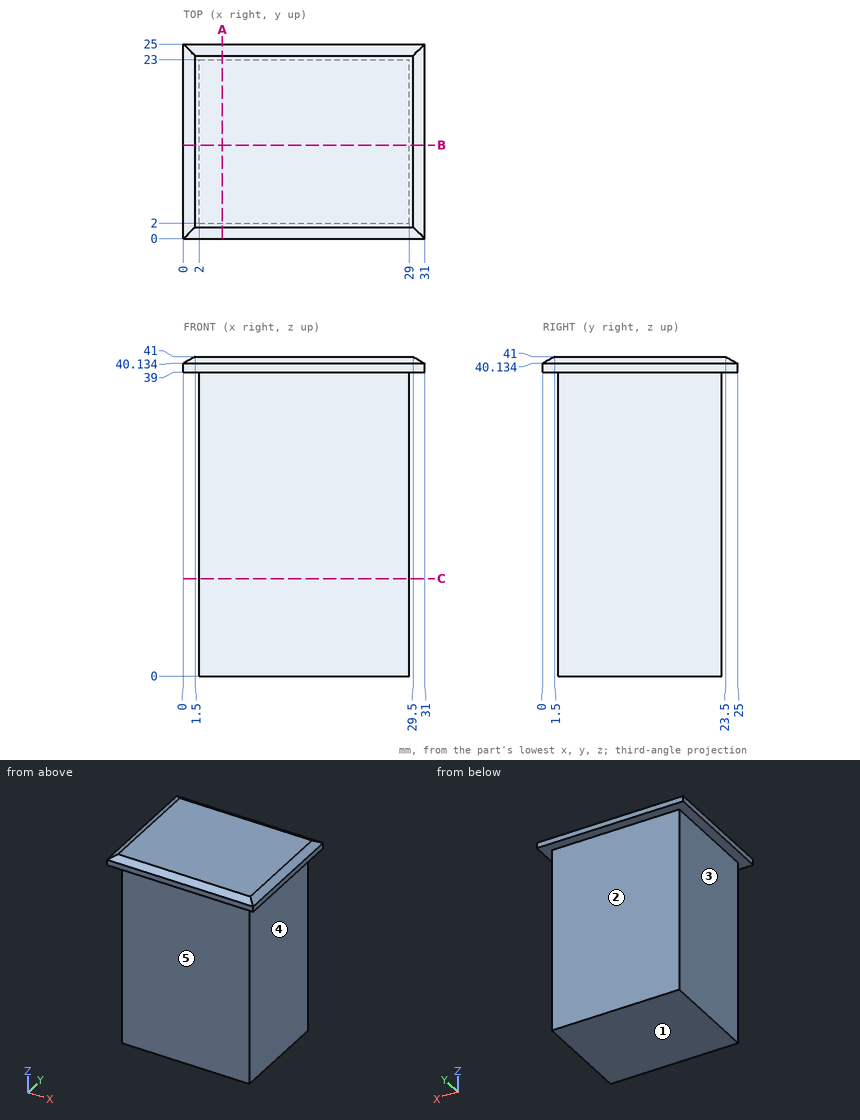
Check sheet for the drawn part. Datum: minimum x, y, z corner. Units: mm. A direction names the side the tool comes from. Round coordinates to 2 decimals unless told otherwise and drop trailing zeros. Loops run counter-clockwise (first coordinate to the right, second up) from the corner with the lowest first, then second, coordinate; pieces in that order, holes last. Notation, with made-up numbers: (-23.75, 63) -> (28.25, 63) arc R20 ccw to (28.25, 97) -> close; hole circle Ø4 at (-27.75, -9). An arc over 180 degrees is marked (long way). Put each result on its own line as item: value. Start each with the question number.
1. Section check B-B (y = 12). Enter the section's corners in (x, z), plus the area to 3 significant figures.
2. Access from +Z, -Z, +X, -X, +Y, -Y to the whole of each face (thin tool, end or side, straight path). Record for the marked faces 1, 2, 3, 4 and 5.
3. Gauge pin test, flat ends, axial feed: pin 1 (3 mm diameter, centred on x = 18.5, z = 22, fed in from +Y); pin 2 (13.5 mm diameter, centred on x = 21, z = 13.5, fed in from -Y); pin 3 (3 mm diameter, centred on y = 18, z = 32, fed in from +X). Record the tip position at first contact, or that the pin passes through.
4. Section check A-A (x = 5). Enter the section's corners in (y, z), plus the area to 3 significant figures.
5. Section check C-C (z = 12.5). Enter the section's corners in (x, y).
6. Scan lines: probe 1 along X at (y, z) = (11, 29.5); probe 2 along Y at (x, z) = (20.5, 35); probe 3 along Z at (x, y) = (10, 23.25). Record each from-to range of solid material in increasing order.
Findings:
1. outline: (0, 39) -> (2, 39) -> (2, 0) -> (29, 0) -> (29, 39) -> (31, 39) -> (31, 40.13) -> (29.5, 41) -> (1.5, 41) -> (0, 40.13) -> close
1. area: 1,110 mm^2
2. face 1: -Z, +X, -X, +Y, -Y
2. face 2: -Z, +X, -X, +Y
2. face 3: -Z, -X, +Y, -Y
2. face 4: -Z, +X, +Y, -Y
2. face 5: -Z, +X, -X, -Y
3. pin 1: stops at y = 23
3. pin 2: stops at y = 2
3. pin 3: stops at x = 29
4. outline: (0, 39) -> (2, 39) -> (2, 0) -> (23, 0) -> (23, 39) -> (25, 39) -> (25, 40.13) -> (23.5, 41) -> (1.5, 41) -> (0, 40.13) -> close
4. area: 868 mm^2
5. outline: (2, 2) -> (29, 2) -> (29, 23) -> (2, 23) -> close
6. probe 1: x = 2 to 29
6. probe 2: y = 2 to 23
6. probe 3: z = 39 to 41
